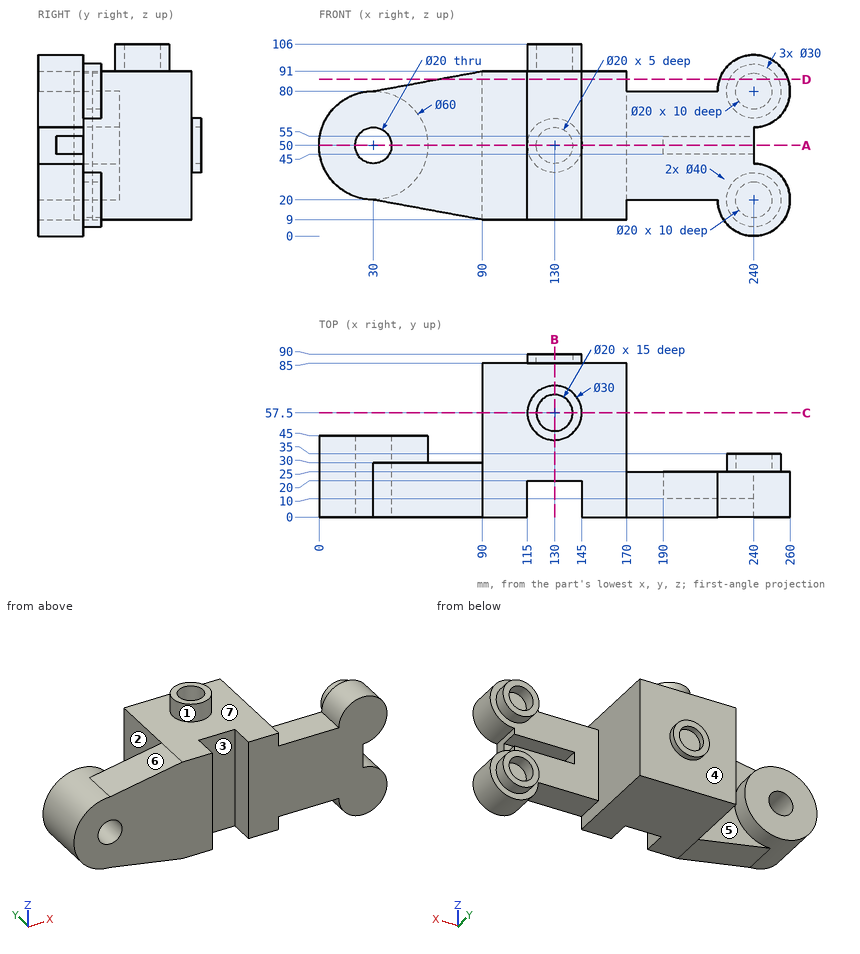
Can you work these out from the drawing? Everything is in mm from the part's minimum corner. A direction names the side the tool comes from. Round coordinates to 2 decimals unless told otherwise and drop trailing zeros. Loops run counter-clockwise (first coordinate to the right, second up) from the corner with the lowest first, then second, coordinate; pieces in that order, holes last. Notation, with made-up numbers: (-11.5, 38) - (35.5, 38) arc R19 cw to (35.5, 69) - close; hole circle Ø9 at (18, 10). An arc over 180 degrees is marked (long way). Answer in a Markdown table with one row per item. Add a question column.
(1) I need wall thicknesses on line 1 along Z through (x, y) = (248.5, 32); line 2 along Y through (x, z) = (130, 97.75); line 3 along Z through (x, y) = (30, 29). Which ranges of each line are inside material? Lowest first, please.
(2) If we section it at A-A (z = 50): Please give me the cut outline in (x, y).
(3) If we mould it in two halves opening along X, with no side actions, what happens to the marked faces 5, 6 and 7? For each: pulls with the +X half, pulls with the -X half, needs draft (parallel to the pull), parting line crosses it, or undercut.
(4) If we section it at C-C (y = 57.5): Please give me the cut outline in (x, z).
(5) I'm going to push flat-ended pins straight in: pin 1 (22 mm diameter, centred on x = 238, z = 19, fed in from +Y); pin 2 (11 mm diameter, centred on y = 20.5, z = 48.5, fed in from +X); pin 3 (2 mm diameter, centred on x = 173.5, z = 31, fed in from +Y). Where does each tip first touch, or does it pass through?
(6) If we section it at D-D (z = 86.5): Please give me the cut outline in (x, y).
(7) For the marked faces 1, 2, 3 and 4, which set-ups out of +Z, -Z, +X, -X, +Y, -Y let a thin tool reach every point of the face, with its end or its side?
(8) If we section it at B-B (x = 130): Please give me the cut outline in (y, z), plus the area to 3 significant figures.
Model answer:
| question | item | result |
|---|---|---|
| 1 | line 1 | z = 7.64 to 14.73, 25.27 to 32.36, 67.64 to 74.73, 85.27 to 92.36 |
| 1 | line 2 | y = 42.5 to 47.5, 67.5 to 72.5 |
| 1 | line 3 | z = 20 to 40, 60 to 80 |
| 2 | outline | (0, 0) - (20, 0) - (20, 45) - (0, 45) - close; (40, 0) - (115, 0) - (115, 20) - (145, 20) - (145, 0) - (240, 0) - (240, 10) - (190, 10) - (190, 25) - (170, 25) - (170, 85) - (145, 85) - (145, 90) - (140, 90) - (140, 85) - (120, 85) - (120, 90) - (115, 90) - (115, 85) - (90, 85) - (90, 30) - (60, 30) - (60, 45) - (40, 45) - close |
| 3 | face 5 | undercut |
| 3 | face 6 | pulls with the -X half |
| 3 | face 7 | needs draft |
| 4 | outline | (90, 9) - (170, 9) - (170, 91) - (145, 91) - (145, 106) - (140, 106) - (140, 91) - (120, 91) - (120, 106) - (115, 106) - (115, 91) - (90, 91) - close |
| 5 | pin 1 | stops at y = 35 |
| 5 | pin 2 | stops at x = 240 |
| 5 | pin 3 | stops at y = 25 |
| 6 | outline | (65.45, 0) - (115, 0) - (115, 20) - (145, 20) - (145, 0) - (170, 0) - (170, 85) - (90, 85) - (90, 30) - (65.45, 30) - close; (221.09, 0) - (258.91, 0) - (258.91, 25) - (253.52, 25) - (253.52, 35) - (247.6, 35) - (247.6, 25) - (232.4, 25) - (232.4, 35) - (226.48, 35) - (226.48, 25) - (221.09, 25) - close |
| 7 | face 1 | +Z |
| 7 | face 2 | +Z, -Z, +Y |
| 7 | face 3 | +Z, -Z, -Y |
| 7 | face 4 | +Y |
| 8 | outline | (20, 9) - (85, 9) - (85, 35) - (90, 35) - (90, 40) - (85, 40) - (85, 60) - (90, 60) - (90, 65) - (85, 65) - (85, 91) - (72.5, 91) - (72.5, 106) - (67.5, 106) - (67.5, 91) - (47.5, 91) - (47.5, 106) - (42.5, 106) - (42.5, 91) - (20, 91) - close |
| 8 | area | 5,530 mm² |
